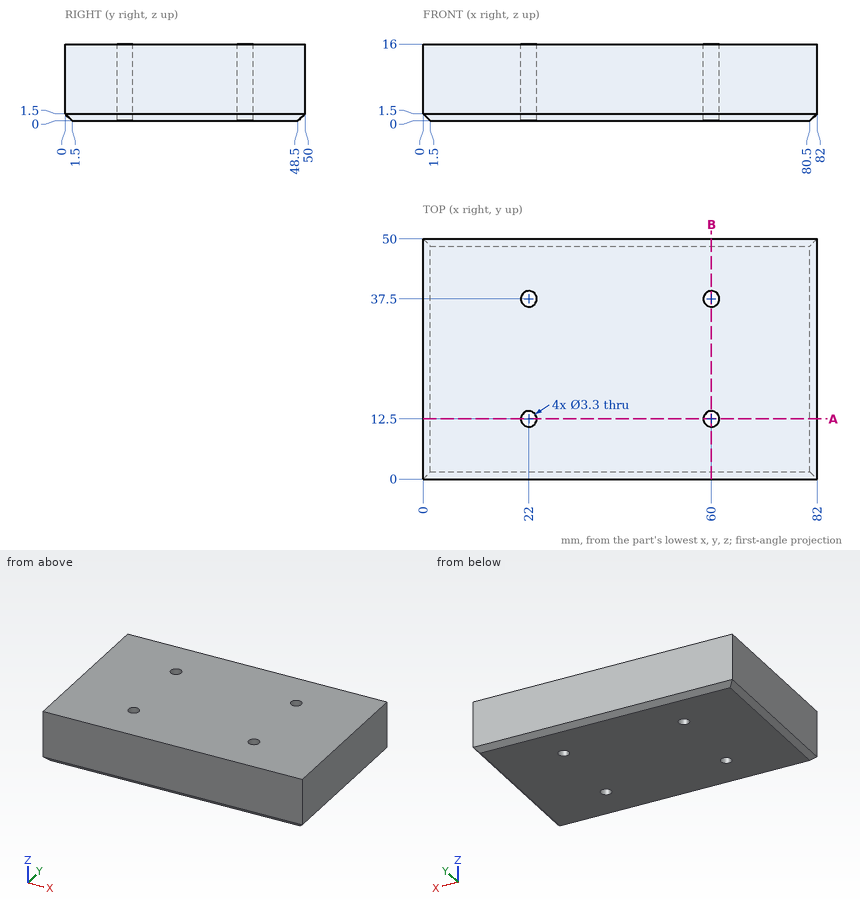
Design review of the part shown in the three views and the two pictorial views. Dimensions are in mm from the part's minimum x, y and z. Round coordinates to 2 decimals unless told otherwise and drop trailing zeros. Order: outer loops, then holes, each group sorted by start corner. A loop starts at its lowest first (then second) coordinate and runs counter-clockwise, first axis right, second up.
(1) Take a section at A-A, the plane y = 12.5. State the section outline as (x, z) points, plus the area to 3 significant figures.
Working result:
outline: (0, 1.5) - (1.5, 0) - (20.35, 0) - (20.35, 16) - (0, 16) - close; (23.65, 0) - (58.35, 0) - (58.35, 16) - (23.65, 16) - close; (61.65, 0) - (80.5, 0) - (82, 1.5) - (82, 16) - (61.65, 16) - close
area: 1,200 mm2
(2) Wall thickness on L1, parallel to Y at x = 60, z = 11.5; L2, parallel to X at y = 12, z = 13.75; L3, parallel to Y at x = 55, z = 1: over which ranges is each line inside the solid? List them lowest first.
Working result:
L1: y = 0 to 10.85, 14.15 to 35.85, 39.15 to 50
L2: x = 0 to 20.43, 23.57 to 58.43, 61.57 to 82
L3: y = 0.5 to 49.5
(3) Take a section at B-B, the plane x = 60. State the section outline as (y, z) points, plus the area to 3 significant figures.
Working result:
outline: (0, 1.5) - (1.5, 0) - (10.85, 0) - (10.85, 16) - (0, 16) - close; (14.15, 0) - (35.85, 0) - (35.85, 16) - (14.15, 16) - close; (39.15, 0) - (48.5, 0) - (50, 1.5) - (50, 16) - (39.15, 16) - close
area: 692 mm2
(4) For P1, Ø2, axis at x = 60, y = 12.5, coming from the +Z side, flat-tipped, find the tip position at first contact; note if it passes through.
Working result:
P1: passes through
